Check sheet for the drawn part. Datum: minimum x, y, z corner. Units: mm. A direction names the side the tool comes from. Give positions to 0.01 mm unless a question says otherwise; leave off trailing zeros. Order: outer loops, then holes, each group sorted by start corner. A loop starts at its lowest first (then second) coordinate and runs counter-clockwise, first axis right, second up.
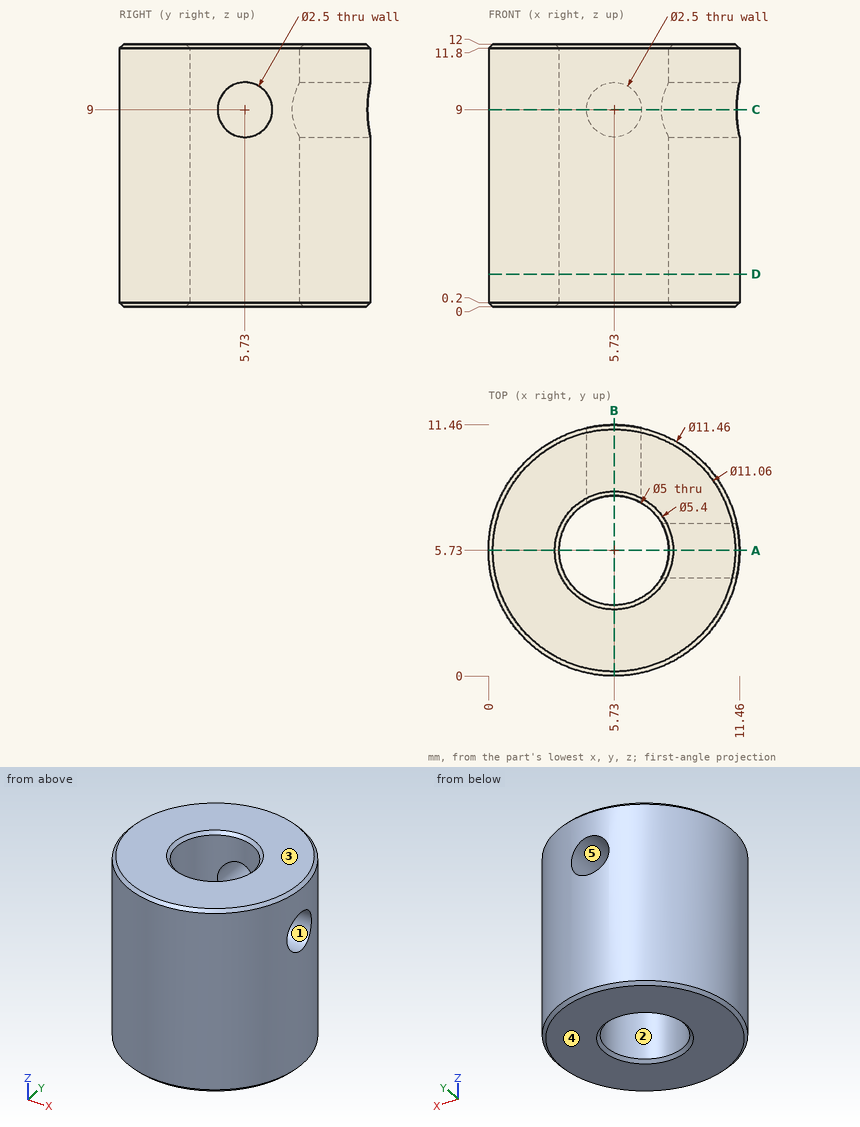
Q1. Sectioned sample at A-A, the plane y = 5.73. Record the cut outline in (x, z), plus the area to 3 significant figures.
Q2. Material ranges on line 1 (Y direction, x = 5.73, z = 6.25); line 2 (X direction, y = 4.25, z = 11); line 3 (Y direction, x = 8.85, z = 9), recorded low to high.
Q3. Sectioned sample at D-D, the plane z = 1.5. Record the cut outline in (x, y).
Q4. Tool access check on the marked faces 1 and 2. Record the directions out of +Z, -Z, +X, -X, +Y, -Y that give a thin tool (end or side, any length) a straight path to the whole face; none if there is none.
Q5. Draft check along Z on the marked faces 3, 4 and 5. Enter one of: pulls with the +Z half, pulls with the -Z half, needs draft (parallel to the pull), parting line crosses it, or undercut.
Q6. Go/stop test with flat-tipped pins: P1, Ø1.5, axis at x = 4.5, z = 9.5, coming from the -Y side; P2, Ø4, axis at x = 2, z = 4.5, coming from the +Y side; P3, Ø1, axis at x = 3.5, z = 4.5, coming from the -Y side. Record where each tip stops, or that it passes through.
Q7. Sectioned sample at C-C, the plane z = 9. Record the cut outline in (x, y), plus the area to 3 significant figures.
Filled in:
1. outline: (0, 0.2) - (0.2, 0) - (3.03, 0) - (3.23, 0.2) - (3.23, 11.8) - (3.03, 12) - (0.2, 12) - (0, 11.8) - close; (8.23, 0.2) - (8.43, 0) - (11.26, 0) - (11.46, 0.2) - (11.46, 7.75) - (8.23, 7.75) - close; (8.23, 10.25) - (11.46, 10.25) - (11.46, 11.8) - (11.26, 12) - (8.43, 12) - (8.23, 11.8) - close
1. area: 69.3 mm2
2. line 1: y = 0 to 3.23, 8.23 to 11.46
2. line 2: x = 0.19 to 3.72, 7.74 to 11.27
2. line 3: y = 0.92 to 4.48, 6.98 to 10.54
3. outline: circle Ø11.46 at (5.73, 5.73); hole circle Ø5 at (5.73, 5.73)
4. face 1: +X
4. face 2: +Z, -Z
5. face 3: pulls with the +Z half
5. face 4: pulls with the -Z half
5. face 5: undercut
6. P1: stops at y = 0.02
6. P2: stops at y = 11.19
6. P3: stops at y = 0.27
7. outline: (4.48, 7.9) - (4.48, 11.32) arc R5.73 ccw (long way) to (11.32, 4.48) - (7.9, 4.48) arc R2.5 cw (long way) to start; (6.98, 7.9) arc R2.5 cw to (7.9, 6.98) - (11.32, 6.98) arc R5.73 ccw to (6.98, 11.32) - close
7. area: 67.0 mm2
